Geometry check sheet. Reference: the model listing, model coordinates, mm. Coordinates: 2 decimals unless noted, no trailing zeros. Write each loop counter-clockwise with the first axis right and the second up, starting at its lowest first coordinate (ties: lowest second). Pieces come first, ordered by that corner, then holes. Notation, with made-up numbers: (-31, -10) - (26, -10) arc R16 ccw to (26, -2) - close; hole circle Ø9 at (82.25, 44). An arc over 180 degrees is marked (long way). Answer as a JSON object with one key per item and string values. Group by question number.
from build123d import *

# Parameters (mm, degrees)
EXTRUDE_1_DEPTH = 14


with BuildPart() as part:
    # 草图1 → 凸台-拉伸1 (new body)
    with BuildSketch(Plane.XY):
        Polygon((0, 0), (0, 85), (50, 85), (50, 50), (35.5, 0), align=None)
    extrude(amount=EXTRUDE_1_DEPTH)


solid = part.part
(1) Material ranges on L1, parallel to X at y = 4.5, z = 6.25 (3 decimals); L2, parallel to X at y = 6.5, z = 2.25 (3 decimals), recorded low to high. Write a range as [from, to].
(2) Section check B-B (y = 28). Record the cut outline in (x, z), and give its area (3 significant figures).
(3) Section check A-A (z = 5.25). Record the cut outline in (x, y).
(4) Section check C-C (x = 42.5). Record the cut outline in (y, z), and give its area (3 significant figures).
Conclusion:
{
 "1": {"L1": "x = [0, 36.805]", "L2": "x = [0, 37.385]"},
 "2": {"outline": "(0, 0) - (43.62, 0) - (43.62, 14) - (0, 14) - close", "area": "611 mm^2"},
 "3": {"outline": "(0, 0) - (35.5, 0) - (50, 50) - (50, 85) - (0, 85) - close"},
 "4": {"outline": "(24.14, 0) - (85, 0) - (85, 14) - (24.14, 14) - close", "area": "852 mm^2"}
}
